For this review, take the finished solid that the model builds, in its own axes (mm). A direction names the side the tool comes from. Give positions to 0.01 mm unless a question says otherwise; leave off trailing zeros. Loops run counter-clockwise (first coordinate to the right, second up) from the corner with the lowest first, then second, coordinate; pieces in that order, holes last. Notation, with made-up numbers: (11, -4.75) - (57, -4.75) arc R13 ccw to (57, 0.25) - close; hole circle Ø2 at (52.5, 22). An arc over 180 degrees is marked (long way). Answer in a Markdown table with one row per item.
```python
from build123d import *

# Parameters (mm, degrees)
SKETCH1_W           = 198
SKETCH1_H           = 98
BOSS_EXTRUDE1_DEPTH = 22
SKETCH2_R           = 5
BOSS_EXTRUDE2_DEPTH = 30
SKETCH3_R           = 5
BOSS_EXTRUDE3_DEPTH = 2
SKETCH4_R           = 2.5
BOSS_EXTRUDE4_DEPTH = 2


with BuildPart() as part:
    # Sketch1 → Boss-Extrude1 (new body)
    with BuildSketch(Plane(origin=(0, 0, 0), x_dir=(1, 0, 0), z_dir=(0, 1, 0))):
        Rectangle(SKETCH1_W, SKETCH1_H)
    extrude(amount=BOSS_EXTRUDE1_DEPTH)

    # Sketch2 → Boss-Extrude2 (add)
    with BuildSketch(Plane(origin=(99, 0, 0), x_dir=(0, 0, -1), z_dir=(1, 0, 0))):
        with Locations(Location((0, 9.760048185, 0), (0, 0, 180))):
            Circle(SKETCH2_R)
    extrude(amount=BOSS_EXTRUDE2_DEPTH)

    # Sketch3 → Boss-Extrude3 (add)
    with BuildSketch(Plane(origin=(0, 22, 0), x_dir=(1, 0, 0), z_dir=(0, 1, 0))):
        with Locations(Location((61, 0, 0), (0, 0, 90))):
            Circle(SKETCH3_R)
    extrude(amount=BOSS_EXTRUDE3_DEPTH)

    # Sketch4 → Boss-Extrude4 (add)
    with BuildSketch(Plane(origin=(99, 0, 0), x_dir=(0, 0, -1), z_dir=(1, 0, 0))):
        with Locations(Location((23, 10.330807158, 0), (0, 0, 180))):
            Circle(SKETCH4_R)
        with Locations(Location((-23, 11.325219915, 0), (0, 0, 180))):
            Circle(SKETCH4_R)
    extrude(amount=BOSS_EXTRUDE4_DEPTH)


solid = part.part
```
1. Wall thickness on line 1 (X direction, y = 17.25, z = 17); line 2 (Y direction, x = 88, z = -5): over which ranges is each line inside the solid? List them lowest first. Write a range as [from, to].
Values:
| item | result |
|---|---|
| line 1 | x = [-99, 99] |
| line 2 | y = [0, 22] |
2. We need section A-A, the plane z = -23. Give the boundary of the cut face in (x, y), and give its area (3 significant figures).
Values:
| item | result |
|---|---|
| outline | (-99, 0) - (99, 0) - (99, 7.83) - (101, 7.83) - (101, 12.83) - (99, 12.83) - (99, 22) - (-99, 22) - close |
| area | 4,370 mm^2 |
3. We need section C-C, the plane z = 0. Give the boundary of the cut face in (x, y), and give its area (3 significant figures).
Values:
| item | result |
|---|---|
| outline | (-99, 0) - (99, 0) - (99, 4.76) - (129, 4.76) - (129, 14.76) - (99, 14.76) - (99, 22) - (66, 22) - (66, 24) - (56, 24) - (56, 22) - (-99, 22) - close |
| area | 4,680 mm^2 |
4. Clearance check with flat-ended pins moving along their axes: pin 1 (3 mm diameter, centred on y = 16.5, z = -8, fed in from +X); pin 2 (2.5 mm diameter, centred on y = 10, z = -22.5, fed in from +X). State where each tip first meets the part, or that it passes through.
Values:
| item | result |
|---|---|
| pin 1 | stops at x = 99 |
| pin 2 | stops at x = 101 |
5. We need section B-B, the plane x = 61. Give the boundary of the cut face in (y, z), and give its area (3 significant figures).
Values:
| item | result |
|---|---|
| outline | (0, -49) - (22, -49) - (22, -5) - (24, -5) - (24, 5) - (22, 5) - (22, 49) - (0, 49) - close |
| area | 2,180 mm^2 |
6. For faces 1 (the face through (101, 11, 23)), 2 (the face through (113.79, 9.54, -4.995)), 3 (the face through (56.043, 22.986, 0.651)), 4 (the face through (61, 24, 0)), 5 (the face through (101, 10, -23)), list the 3-axis set-ups (+Z, -Z, +X, -X, +Y, -Y) from which the entire face can be reached by the end or side of a thin tool; tool diameter is ignored.
Values:
| item | result |
|---|---|
| face 1 | +Z, +X, +Y, -Y |
| face 2 | +X |
| face 3 | +Y |
| face 4 | +Z, -Z, +X, -X, +Y |
| face 5 | -Z, +X, +Y, -Y |
7. We need section D-D, the plane y = 18.25. Give the boundary of the cut face in (x, z).
Values:
| item | result |
|---|---|
| outline | (-99, -49) - (99, -49) - (99, 49) - (-99, 49) - close |
8. Mouldability with a two-part tool opening along Z and no side actions: class faces 6 (the face through (-1, 11, -49)), 7 (the face through (99.986, 10.221, -25.498)), 8 (the face through (-1, 0, -1)), 9 (the face through (99.986, 9.636, 21.157)) as released by +Z, released by -Z, zero draft, split by the parting line, or undercut.
Values:
| item | result |
|---|---|
| face 6 | released by -Z |
| face 7 | undercut |
| face 8 | zero draft |
| face 9 | undercut |
